Read the model definition and answer for the solid it produces. Units are mm, in the model's axes. Face numbers are marked on the shaded views. A direction names the side the tool comes from. Coordinates: 2 decimals unless noted, no trailing zeros. Order: outer loops, then holes, each group sorted by start corner. A loop starts at its lowest first (then second) coordinate and runs counter-clockwise, first axis right, second up. Notation, with made-up numbers: (75.5, 70) - (89.5, 70) arc R12 ccw to (89.5, 91) - close; hole circle Ø8 at (-9.75, 37). An arc over 180 degrees is marked (long way). Write item = value, one per line.
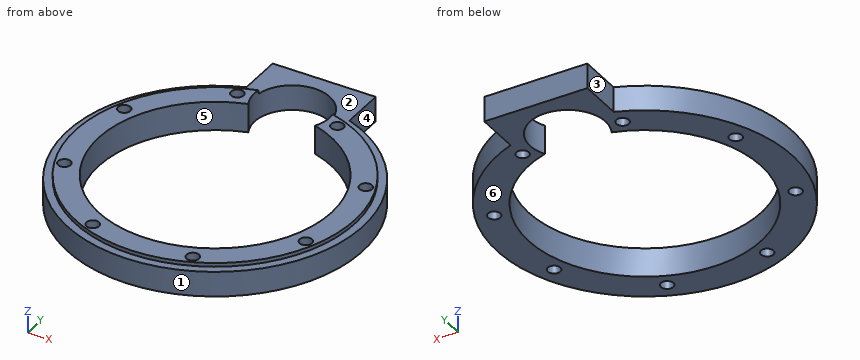
from build123d import *

# Parameters (mm, degrees)
SKETCH_1_R          = 117.5
SKETCH_1_R_2        = 92.5
EXTRUDE_1_DEPTH     = 20
SKETCH_2_W          = 82
SKETCH_2_H          = 52.5
EXTRUDE_2_DEPTH     = 20
SKETCH_7_R          = 111
SKETCH_7_R_2        = 92.5
EXTRUDE_3_DEPTH     = 3
SKETCH_3_R          = 30
CUT_EXTRUDE_1_DEPTH = 189.043213119
HOLE_WIZARD_M8_1_D  = 10


with BuildPart() as part:
    # 草图1 → 凸台-拉伸1 (new body)
    with BuildSketch(Plane.XY):
        Circle(SKETCH_1_R)
        Circle(SKETCH_1_R_2, mode=Mode.SUBTRACT)
    extrude(amount=EXTRUDE_1_DEPTH)

    # 草图2 → 凸台-拉伸2 (add, through all)
    with BuildSketch(Plane.XY.offset(20)):
        with Locations((0, 118.75)):
            Rectangle(SKETCH_2_W, SKETCH_2_H)
    extrude(amount=-EXTRUDE_2_DEPTH)

    # 草图7 → 凸台-拉伸3 (add)
    with BuildSketch(Plane.XY.offset(20)):
        Circle(SKETCH_7_R)
        Circle(SKETCH_7_R_2, mode=Mode.SUBTRACT)
    extrude(amount=EXTRUDE_3_DEPTH)

    # 草图3 → 切除-拉伸1 (cut, through all)
    with BuildSketch(Plane(origin=(0, 0, 0), x_dir=(-1, 0, 0), z_dir=(0, 0, -1))):
        with Locations((0, 102.5)):
            Circle(SKETCH_3_R)
    extrude(amount=-CUT_EXTRUDE_1_DEPTH, mode=Mode.SUBTRACT)

    # M8 间隙孔1 (through all)
    with Locations(Plane(origin=(0, 0, 0), x_dir=(-1, 0, 0), z_dir=(0, 0, -1))):
        with Locations((-39.799076966, 96.083471381), (-96.083471381, 39.799076966), (-96.083471381, -39.799076966), (-39.799076966, -96.083471381), (39.799076966, -96.083471381), (96.083471381, -39.799076966), (96.083471381, 39.799076966), (39.799076966, 96.083471381)):
            Hole(HOLE_WIZARD_M8_1_D / 2)


solid = part.part
1) The part is cut by section C-C (z = 14.75). Count the separate pieces of the cut face and the enclosed holes in it, and give its area (3 significant figures).
Returned:
separate_pieces = 1
enclosed_holes = 9
area = 16,200 mm^2
2) The part is cut by section B-B (x = 67). Determine the outline of the cut face in (y, z) (3 decimals), and give its area (3 significant figures).
Returned:
outline = (-96.526, 0) - (-63.775, 0) - (-63.775, 23) - (-88.499, 23) - (-88.499, 20) - (-96.526, 20) - close; (63.775, 0) - (96.526, 0) - (96.526, 20) - (88.499, 20) - (88.499, 23) - (63.775, 23) - close
area = 1,460 mm^2
3) The part is cut by section D-D (x = -11.5). Determine the outline of the cut face in (y, z).
Returned:
outline = (-116.94, 0) - (-91.78, 0) - (-91.78, 23) - (-110.4, 23) - (-110.4, 20) - (-116.94, 20) - close; (130.21, 0) - (145, 0) - (145, 20) - (130.21, 20) - close
4) Determine the mould class of the marked faces 3, 4, 5 and 6 for opening direction X: pulls with the +X half, pulls with the -X half, needs draft (parallel to the pull), parting line crosses it, or undercut.
Returned:
face_3 = pulls with the -X half
face_4 = pulls with the +X half
face_5 = undercut
face_6 = needs draft
5) The part is cut by section A-A (y = 0). Determine the outline of the cut face in (x, z), and give its area (3 significant figures).
Returned:
outline = (-117.5, 0) - (-92.5, 0) - (-92.5, 23) - (-111, 23) - (-111, 20) - (-117.5, 20) - close; (92.5, 0) - (117.5, 0) - (117.5, 20) - (111, 20) - (111, 23) - (92.5, 23) - close
area = 1,110 mm^2
6) Flat-ended cylindrical pins translate along their axes: pin 1 Ø2 at (y, z) = (116.5, 12) entering from +X; pin 2 Ø8 at (y, z) = (-38, 8.5) entering from +X; pin 3 Ø10 at (y, z) = (93.5, 9.5) entering from -X. Find the tip coordinate at first contact, or state that the pin passes through.
Returned:
pin_1 = 41
pin_2 = 112.47
pin_3 = -77.29
7) For the marked faces 1 and 2, determine the directions among +Z, -Z, +X, -X, +Y, -Y from which every point of the face is accessible in a straight line to the end or side of a thin tool.
Returned:
face_1 = +Z, -Z
face_2 = +Z
8) Straight lines are drawn through the part: line 1 along Y through (x, z) = (-95.5, 18.5); line 2 along Y through (x, z) = (0, 13.25); line 3 along X through (y, z) = (-7, 4.5). For each, find the intervals that lie inside material, in ascending order. Write a range as from..to.
Returned:
line_1 = -68.45..-44.76, -34.83..34.83, 44.76..68.45
line_2 = -117.5..-92.5, 132.5..145
line_3 = -117.29..-92.23, 92.23..117.29
